Design review of the part built by this model. Coordinates are the model's own, in mm. A direction names the side the tool comes from. Coordinates: 2 decimals unless noted, no trailing zeros. Write each loop counter-clockwise with the first axis right and the second up, starting at its lowest first coordinate (ties: lowest second). Pieces come first, ordered by that corner, then holes.
Q1. For faces 1 (the flat face through (17, -24, 5)), 2 (the flat face through (-17, -24, 5)), 3 (the flat face through (-17, 24, 5)), 4 (the flat face through (17, 24, 5)), list the 3-axis set-ups (+Z, -Z, +X, -X, +Y, -Y) from which the entire face can be reached by the end or side of a thin tool; tool diameter is ignored.
Q2. For L1, parallel to Y at x = 21, z = 1; L2, parallel to X at y = 30, z = 8, list the stretches that pass through material, from the lowest coordinate up.
Q3. Take a section at A-A, the plane z = 5. Write out the cut boundary in (x, y).
Q4. For pin 1 Ø3 at (x, z) = (-17, 7) entering from +Y; pin 2 Ø5 at (x, z) = (-15.5, 3.5) entering from -Y; pin 3 Ø5 at (y, z) = (30, 4) entering from +X, all flat-tipped, find the tip position at first contact; note any pin that passes through.
Q5. Take a section at B-B, the plane x = -11. Write out the cut boundary in (y, z), plus the area to 3 significant figures.
from build123d import *

# Parameters (mm, degrees)
SKETCH1_W           = 48
SKETCH1_H           = 68
BOSS_EXTRUDE1_DEPTH = 10
SKETCH2_W           = 28
SKETCH2_H           = 20
CUT_EXTRUDE1_DEPTH  = 10


with BuildPart() as part:
    # Sketch1 → Boss-Extrude1 (new body)
    with BuildSketch(Plane.XY):
        Rectangle(SKETCH1_W, SKETCH1_H)
    extrude(amount=BOSS_EXTRUDE1_DEPTH)

    # Sketch2 → Cut-Extrude1 (cut)
    with BuildSketch(Plane.XY.offset(10)):
        with Locations((-24, 34)):
            Rectangle(SKETCH2_W, SKETCH2_H)
        with Locations((24, 34)):
            Rectangle(SKETCH2_W, SKETCH2_H)
        with Locations((24, -34)):
            Rectangle(SKETCH2_W, SKETCH2_H)
        with Locations((-24, -34)):
            Rectangle(SKETCH2_W, SKETCH2_H)
    extrude(amount=-CUT_EXTRUDE1_DEPTH, mode=Mode.SUBTRACT)


solid = part.part
Responses:
1. face 1: +Z, -Z, +X, -Y
1. face 2: +Z, -Z, -X, -Y
1. face 3: +Z, -Z, -X, +Y
1. face 4: +Z, -Z, +X, +Y
2. L1: y = -24 to 24
2. L2: x = -10 to 10
3. outline: (-24, -24) - (-10, -24) - (-10, -34) - (10, -34) - (10, -24) - (24, -24) - (24, 24) - (10, 24) - (10, 34) - (-10, 34) - (-10, 24) - (-24, 24) - close
4. pin 1: stops at y = 24
4. pin 2: stops at y = -24
4. pin 3: stops at x = 10
5. outline: (-24, 0) - (24, 0) - (24, 10) - (-24, 10) - close
5. area: 480 mm2
